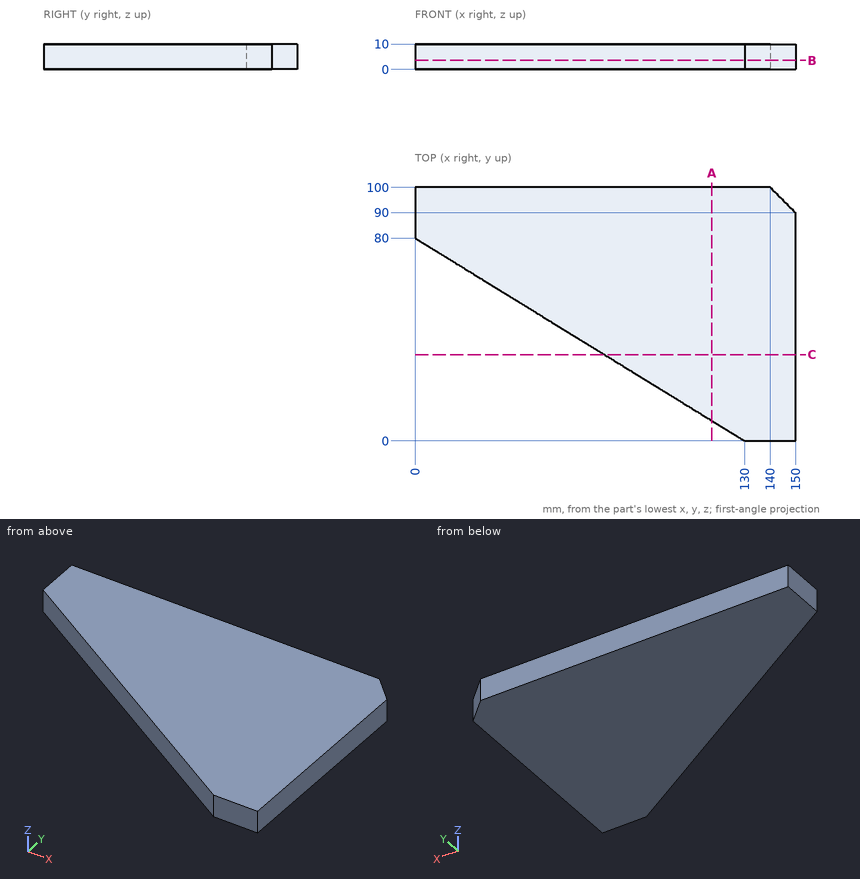
Geometry: see drawing. Coordinates: mm, zero at the bounding-box minimum. Coordinates: 2 decimals unless noted, no trailing zeros. Loops run counter-clockwise (first coordinate to the right, second up) from the corner with the lowest first, then second, coordinate; pieces in that order, holes last.
(1) Section C-C on y = 34. Return the cut outline in (x, z).
(2) Section A-A on x = 117. Return the cut outline in (y, z).
(3) Material intervals for probe 1 along X at (y, z) = (65, 8.25) (3 decimals); probe 2 along X at (y, z) = (62.5, 6); probe 3 along Y at (x, z) = (80, 0.5), sorted ascending.
(4) Section B-B on z = 3.5. Return the cut outline in (x, y), then the cut area to 3 significant figures.
(5) First-contact query: pin 1 Ø6 at (y, z) = (72.5, 3.5) entering from -X; pin 2 Ø1 at (x, z) = (44.5, 2) entering from -Y. Flat tips, straight axial feed; report the tip coordinate or a pass-through.
Data:
1. outline: (74.75, 0) - (150, 0) - (150, 10) - (74.75, 10) - close
2. outline: (8, 0) - (100, 0) - (100, 10) - (8, 10) - close
3. probe 1: x = 24.375 to 150
3. probe 2: x = 28.44 to 150
3. probe 3: y = 30.77 to 100
4. outline: (0, 80) - (130, 0) - (150, 0) - (150, 90) - (140, 100) - (0, 100) - close
4. area: 9,750 mm2
5. pin 1: stops at x = 7.31
5. pin 2: stops at y = 52.31
